Model file for the job. Use its own axes, mm. Round coordinates to 2 decimals unless told otherwise and drop trailing zeros. Loops run counter-clockwise (first coordinate to the right, second up) from the corner with the lowest first, then second, coordinate; pieces in that order, holes last. Notation, with made-up numbers: M 59,34.25 L 108,34.25 A37 ccw 108,73.25 Z; hole C 46.5,-15 d3. An arc over 180 degrees is marked long. Use a Markdown table: item, result. Add a question column.
Item 1: Saw through at A-A on z = -235. Write the cut outline in (x, y).
Item 2: Pin check, flat tips, straight feed: P1, Ø6, axis at y = 19, z = -166, coming from the +X side; P2, Ø6.5, axis at x = 15, z = -190, coming from the +Y side; P3, Ø3.5, axis at y = 10, z = 184.5, coming from the -X side. Stop position of each tip, or through.
Item 3: Wall check: L1, parallel to X at y = 3, z = -190; L2, parallel to Y at x = 17.5, z = 280; L3, parallel to X at y = 5.5, z = 241. Give the ranges that are in metal, low to high. Write a range as from..to.
Item 4: Two-plate mould, pull along Y, no slides. Class faces 1 (the flat face through (0, 0, 6)), 2 (the cylindrical face through (0, 33, 6)), 3 (the flat face through (0, 13, 435)): +Y half, -Y half, draft (parallel to the pull), parting line (faces both ways), or undercut.
```python
from build123d import *

# Parameters (mm, degrees)
EXTRUDE_1_DEPTH                  = 435
EXTRUDE_2_DEPTH                  = 870
HOLE_WIZARD_5_5_5_5_1_AT_2_COUNT = 2
HOLE_WIZARD_5_5_5_5_1_AT_2_PITCH = 30
PATTERN_LINEAR_1_COUNT           = 6
PATTERN_LINEAR_1_PITCH           = 150


with BuildPart() as part:
    # 草图1 → 凸台-拉伸1 (new, symmetric)
    with BuildSketch(Plane.XY):
        with BuildLine():
            Line((-9.25, 11.7), (-9.25, 5))
            Line((-9.25, 5), (-20, 5))
            Line((-20, 5), (-20, 0))
            Line((-20, 0), (20, 0))
            Line((20, 0), (20, 5))
            Line((20, 5), (9.25, 5))
            Line((9.25, 5), (9.25, 11.7))
            Line((9.25, 11.7), (9.11850775, 11.7))
            Line((9.11850775, 11.7), (4, 17.8))
            Line((4, 17.8), (3.487119155, 17.8))
            ThreePointArc((3.487119155, 17.8), (0, 17), (-3.487119155, 17.8))
            Line((-3.487119155, 17.8), (-4, 17.8))
            Line((-4, 17.8), (-9.11850775, 11.7))
            Line((-9.11850775, 11.7), (-9.25, 11.7))
        make_face()
    extrude(amount=EXTRUDE_1_DEPTH, both=True)

    # 草图2 → 凸台-拉伸2 (add)
    with BuildSketch(Plane.XY.offset(435)):
        with BuildLine():
            ThreePointArc((3.487119155, 17.8), (0, 33), (-3.487119155, 17.8))
            ThreePointArc((-3.487119155, 17.8), (0, 17), (3.487119155, 17.8))
        make_face()
    extrude(amount=-EXTRUDE_2_DEPTH)

    # 草图3 → Ø5.5 (5.5) 直径孔1 (revolve, cut)
    with BuildSketch(Plane(origin=(15, 5, 410), x_dir=(0, 0, 1), z_dir=(1, 0, 0))):
        Polygon((0, 0), (0, 17.19771324), (2.75, 15.61), (2.75, 0), align=None)
    hole_wizard_5_5_5_5_1 = revolve(axis=Axis((15, 11.35, 410), (0, -1, 0)), mode=Mode.SUBTRACT)

    # Ø5.5 (5.5) 直径孔1 at 2: Ø5.5 (5.5) 直径孔1 ×2
    with Locations(*[(-i * HOLE_WIZARD_5_5_5_5_1_AT_2_PITCH, 0, 0) for i in range(1, HOLE_WIZARD_5_5_5_5_1_AT_2_COUNT)]):
        add(hole_wizard_5_5_5_5_1, mode=Mode.SUBTRACT)

    # 阵列(线性)1: Ø5.5 (5.5) 直径孔1 ×6
    with Locations(*[(0, 0, -i * PATTERN_LINEAR_1_PITCH) for i in range(1, PATTERN_LINEAR_1_COUNT)]):
        add(hole_wizard_5_5_5_5_1, mode=Mode.SUBTRACT)

    # 阵列(线性)1 copy 1 sketch → 阵列(线性)1 copy 1 (revolve, cut)
    with BuildSketch(Plane(origin=(-15, 5, 260), x_dir=(0, 0, 1), z_dir=(1, 0, 0))):
        Polygon((0, 0), (0, 17.19771324), (2.75, 15.61), (2.75, 0), align=None)
    revolve(axis=Axis((-15, 11.35, 260), (0, -1, 0)), mode=Mode.SUBTRACT)

    # 阵列(线性)1 copy 2 sketch → 阵列(线性)1 copy 2 (revolve, cut)
    with BuildSketch(Plane(origin=(-15, 5, 110), x_dir=(0, 0, 1), z_dir=(1, 0, 0))):
        Polygon((0, 0), (0, 17.19771324), (2.75, 15.61), (2.75, 0), align=None)
    revolve(axis=Axis((-15, 11.35, 110), (0, -1, 0)), mode=Mode.SUBTRACT)

    # 阵列(线性)1 copy 3 sketch → 阵列(线性)1 copy 3 (revolve, cut)
    with BuildSketch(Plane(origin=(-15, 5, -40), x_dir=(0, 0, 1), z_dir=(1, 0, 0))):
        Polygon((0, 0), (0, 17.19771324), (2.75, 15.61), (2.75, 0), align=None)
    revolve(axis=Axis((-15, 11.35, -40), (0, -1, 0)), mode=Mode.SUBTRACT)

    # 阵列(线性)1 copy 4 sketch → 阵列(线性)1 copy 4 (revolve, cut)
    with BuildSketch(Plane(origin=(-15, 5, -190), x_dir=(0, 0, 1), z_dir=(1, 0, 0))):
        Polygon((0, 0), (0, 17.19771324), (2.75, 15.61), (2.75, 0), align=None)
    revolve(axis=Axis((-15, 11.35, -190), (0, -1, 0)), mode=Mode.SUBTRACT)

    # 阵列(线性)1 copy 5 sketch → 阵列(线性)1 copy 5 (revolve, cut)
    with BuildSketch(Plane(origin=(-15, 5, -340), x_dir=(0, 0, 1), z_dir=(1, 0, 0))):
        Polygon((0, 0), (0, 17.19771324), (2.75, 15.61), (2.75, 0), align=None)
    revolve(axis=Axis((-15, 11.35, -340), (0, -1, 0)), mode=Mode.SUBTRACT)


solid = part.part
```
Entries:
| question | item | result |
|---|---|---|
| 1 | outline | M -20,0 L 20,0 L 20,5 L 9.25,5 L 9.25,11.7 L 9.12,11.7 L 4,17.8 L 3.49,17.8 A8 ccw long -3.49,17.8 L -4,17.8 L -9.12,11.7 L -9.25,11.7 L -9.25,5 L -20,5 Z |
| 2 | P1 | x = 7.42 |
| 2 | P2 | y = 5 |
| 2 | P3 | x = -9.25 |
| 3 | L1 | -20..-17.75, -12.25..12.25, 17.75..20 |
| 3 | L2 | 0..5 |
| 3 | L3 | -9.25..9.25 |
| 4 | face 1 | -Y half |
| 4 | face 2 | undercut |
| 4 | face 3 | draft |
